from build123d import *

# Parameters (mm, degrees)
SKETCH1_R           = 9
BOSS_EXTRUDE1_DEPTH = 2
SKETCH2_R           = 5.85
BOSS_EXTRUDE2_DEPTH = 46
SKETCH4_R           = 5.35
BOSS_EXTRUDE3_DEPTH = 1
SKETCH5_R           = 5.85
BOSS_EXTRUDE4_DEPTH = 2
CHAMFER1_SIZE       = 1


with BuildPart() as part:
    # Sketch1 → Boss-Extrude1 (new body)
    with BuildSketch(Plane.XY):
        Circle(SKETCH1_R)
    extrude(amount=BOSS_EXTRUDE1_DEPTH)

    # Sketch2 → Boss-Extrude2 (add)
    with BuildSketch(Plane.XY.offset(2)):
        Circle(SKETCH2_R)
    extrude(amount=BOSS_EXTRUDE2_DEPTH)

    # Sketch4 → Boss-Extrude3 (add)
    with BuildSketch(Plane.XY.offset(48)):
        Circle(SKETCH4_R)
    extrude(amount=BOSS_EXTRUDE3_DEPTH)

    # Sketch5 → Boss-Extrude4 (add)
    with BuildSketch(Plane.XY.offset(49)):
        Circle(SKETCH5_R)
    extrude(amount=BOSS_EXTRUDE4_DEPTH)

    # Chamfer1
    chamfer1_edges = [part.edges().sort_by_distance(p)[0] for p in [
        (-5.85, 0, 51),
        (-9, 0, 0),
    ]]
    chamfer(chamfer1_edges, length=CHAMFER1_SIZE)


solid = part.part
The listing builds one solid part. Answer for the finished solid, in the listing's coordinates (mm). A direction names the side the tool comes from. Give positions to 0.01 mm unless a question says otherwise; leave off trailing zeros. Write each loop counter-clockwise with the first axis right and the second up, starting at its lowest first coordinate (ties: lowest second). Pieces come first, ordered by that corner, then holes. Notation, with made-up numbers: (80.5, 84) -> (113.5, 84) arc R23 ccw to (113.5, 107) -> close; hole circle Ø5 at (28, 84.5). An arc over 180 degrees is marked (long way). Use a Markdown table: item, result.
(1) Section A-A, the plane x = 0 is taken. Determine the outline of the cut face in (y, z).
Return value:
| item | result |
|---|---|
| outline | (-9, 1) -> (-8, 0) -> (8, 0) -> (9, 1) -> (9, 2) -> (5.85, 2) -> (5.85, 48) -> (5.35, 48) -> (5.35, 49) -> (5.85, 49) -> (5.85, 50) -> (4.85, 51) -> (-4.85, 51) -> (-5.85, 50) -> (-5.85, 49) -> (-5.35, 49) -> (-5.35, 48) -> (-5.85, 48) -> (-5.85, 2) -> (-9, 2) -> close |
(2) For faces 1 (the flat face through (0, -6, 2)), 2 (the cylindrical face through (-1.172, 8.923, 1.493)), determine the directions among +Z, -Z, +X, -X, +Y, -Y from which every point of the face is accessible in a straight line to the end or side of a thin tool.
Return value:
| item | result |
|---|---|
| face 1 | +Z |
| face 2 | +Z, -Z |
(3) Section C-C, the plane z = 5.5 is taken. Determine the outline of the cut face in (x, y).
Return value:
| item | result |
|---|---|
| outline | circle Ø11.7 at (0, 0) |
(4) Determine the mould class of faces 3 (the cylindrical face through (-1.27, -5.71, 24.68)), 4 (the cylindrical face through (-1.16, -5.223, 48.493)), 5 (the flat face through (0, 0, 51)) for opening direction Z: released by +Z, released by -Z, zero draft, split by the parting line, or undercut.
Return value:
| item | result |
|---|---|
| face 3 | zero draft |
| face 4 | undercut |
| face 5 | released by +Z |
(5) Flat-ended cylindrical pins translate along their axes: P1, Ø8, axis at y = -1.5, z = 17.5, coming from the -X side; P2, Ø1.5, axis at y = -3, z = 6, coming from the -X side; P3, Ø10, axis at x = 7, y = 7, coming from the +Z side; P4, Ø1.5, axis at x = -7, z = 40, coming from the -Y side. Find the tip coordinate at first contact, or state that the pin passes through.
Return value:
| item | result |
|---|---|
| P1 | x = -5.85 |
| P2 | x = -5.4 |
| P3 | z = 50.95 |
| P4 | through |
(6) Find the intervals of material crossed by probe 1 along Z at (x, y) = (-2.25, -5.25); probe 2 along Z at (x, y) = (-7.5, 2.5); probe 3 along Y at (x, z) = (0, 41.5), in increasing order. Write a range as from..to.
Return value:
| item | result |
|---|---|
| probe 1 | 0..48, 49..50.14 |
| probe 2 | 0..2 |
| probe 3 | -5.85..5.85 |
